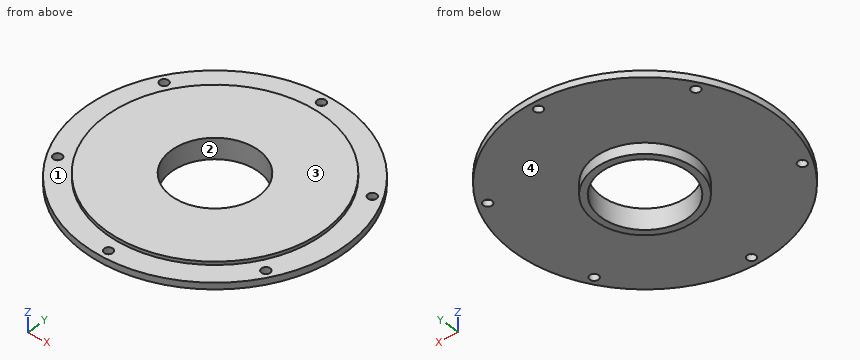
```python
from build123d import *

# Parameters (mm, degrees)
SKETCH2_R          = 2
CUT_EXTRUDE1_DEPTH = 10


with BuildPart() as part:
    # Sketch1 → Revolve1 (revolve)
    with BuildSketch(Plane(origin=(0, 0, 0), x_dir=(1, 0, 0), z_dir=(0, 1, 0)), mode=Mode.PRIVATE) as revolve1_sk:
        Polygon((20, 9.5), (20, 0), (50, 0), (50, 1.5), (60, 1.5), (60, 4.5), (23, 4.5), (23, 9.5), align=None)
    revolve(revolve1_sk.sketch.rotate(Axis((0, 0, -4.956904689), (0, 0, 1)), 180), axis=Axis((0, 0, -4.956904689), (0, 0, 1)))

    # Sketch2 → Cut-Extrude1 (cut)
    with BuildSketch(Plane(origin=(0, 0, -4.5), x_dir=(-1, 0, 0), z_dir=(0, 0, -1))):
        with Locations((0, 56)):
            Circle(SKETCH2_R)
        with Locations((-48.497422612, 28)):
            Circle(SKETCH2_R)
        with Locations((-48.497422612, -28)):
            Circle(SKETCH2_R)
        with Locations((0, -56)):
            Circle(SKETCH2_R)
        with Locations((48.497422612, -28)):
            Circle(SKETCH2_R)
        with Locations((48.497422612, 28)):
            Circle(SKETCH2_R)
    extrude(amount=-CUT_EXTRUDE1_DEPTH, mode=Mode.SUBTRACT)


solid = part.part
```
Check sheet for the modelled part. Datum: model origin and axes. Units: mm. Face numbers are marked on the shaded views. A direction names the side the tool comes from. Coordinates: 2 decimals unless noted, no trailing zeros. Order: outer loops, then holes, each group sorted by start corner. A loop starts at its lowest first (then second) coordinate and runs counter-clockwise, first axis right, second up. Notation, with made-up numbers: (-21.5, -23.75) -> (36.5, -23.75) arc R13 ccw to (36.5, -2.75) -> close; hole circle Ø4 at (87.5, 87). An arc over 180 degrees is marked (long way). Write item = value, one per line. Start each with the question number.
1) Cross-section at C-C (z = -3). Enter the section's corners in (x, y).
2) Material ranges on L1, parallel to Y at x = 0, z = -3.35; L2, parallel to Y at x = 50, z = -4; L3, parallel to Z at x = 1, y = 53, recorded low to high.
3) Cross-section at A-A (y = 0). Enter the section's corners in (x, z).
4) Cross-section at B-B (x = 0). Enter the section's corners in (y, z).
5) Go/stop test with flat-tipped pins: P1, Ø5, axis at x = 10, z = -2, coming from the +Y side; P2, Ø2, axis at y = 17, z = -3.5, coming from the +X side; P3, Ø4.5, axis at x = 0, y = -56, coming from the -Z side; P4, Ø3, axis at y = 1, z = -1, coming from the +X side. Record where each tip stops, or that it passes through.
6) Access from +Z, -Z, +X, -X, +Y, -Y to the whole of each face (thin tool, end or side, straight path). Record for the marked faces 3 and 4.
7) Cross-section at D-D (y = -28). Enter the section's corners in (x, z).
8) Mould release check, pull along Y, two halves, no side actions. Record for the marked faces 1 and 2: +Y half, -Y half, draft (parallel to the pull), parting line (faces both ways), or undercut.
Ans:
q1.outline = circle Ø120 at (0, 0); hole circle Ø4 at (-48.5, -28); hole circle Ø4 at (-48.5, 28); hole circle Ø40 at (0, 0); hole circle Ø4 at (0, -56); hole circle Ø4 at (0, 56); hole circle Ø4 at (48.5, -28); hole circle Ø4 at (48.5, 28)
q2.L1 = -60 to -58, -54 to -20, 20 to 54, 58 to 60
q2.L2 = -33.17 to -29.32, -26.68 to 26.68, 29.32 to 33.17
q2.L3 = -4.5 to -1.5
q3.outline = (-60, -4.5) -> (-23, -4.5) -> (-23, -9.5) -> (-20, -9.5) -> (-20, 0) -> (-50, 0) -> (-50, -1.5) -> (-60, -1.5) -> close; (20, -9.5) -> (23, -9.5) -> (23, -4.5) -> (60, -4.5) -> (60, -1.5) -> (50, -1.5) -> (50, 0) -> (20, 0) -> close
q4.outline = (-60, -4.5) -> (-58, -4.5) -> (-58, -1.5) -> (-60, -1.5) -> close; (-54, -4.5) -> (-23, -4.5) -> (-23, -9.5) -> (-20, -9.5) -> (-20, 0) -> (-50, 0) -> (-50, -1.5) -> (-54, -1.5) -> close; (20, -9.5) -> (23, -9.5) -> (23, -4.5) -> (54, -4.5) -> (54, -1.5) -> (50, -1.5) -> (50, 0) -> (20, 0) -> close; (58, -4.5) -> (60, -4.5) -> (60, -1.5) -> (58, -1.5) -> close
q5.P1 = 59.53
q5.P2 = 57.83
q5.P3 = -4.5
q5.P4 = 60
q6.face_3 = +Z, +X, -X, +Y, -Y
q6.face_4 = -Z
q7.outline = (-53.07, -4.5) -> (-50.5, -4.5) -> (-50.5, -1.5) -> (-53.07, -1.5) -> close; (-46.5, -4.5) -> (46.5, -4.5) -> (46.5, -1.5) -> (41.42, -1.5) -> (41.42, 0) -> (-41.42, 0) -> (-41.42, -1.5) -> (-46.5, -1.5) -> close; (50.5, -4.5) -> (53.07, -4.5) -> (53.07, -1.5) -> (50.5, -1.5) -> close
q8.face_1 = draft
q8.face_2 = undercut
